Geometry check sheet. Reference: the model listing, model coordinates, mm. A direction names the side the tool comes from. Give positions to 0.01 mm unless a question says otherwise; leave off trailing zeros. Loops run counter-clockwise (first coordinate to the right, second up) from the corner with the lowest first, then second, coordinate; pieces in that order, holes last. Notation, with made-up numbers: (79, 88) -> (90, 88) arc R27 cw to (90, 116) -> close; hole circle Ø2 at (31, -14). An arc over 180 degrees is marked (long way). Answer as a JSON object with one key per item and string values.
from build123d import *

# Parameters (mm, degrees)
BASE_BLOCK_PROFILE_W        = 105
BASE_BLOCK_PROFILE_H        = 110
BASE_BLOCK_DEPTH            = 69
FORK_SLOT_PROFILE_W         = 105
FORK_SLOT_PROFILE_H         = 45
FORK_SLOT_CUT_DEPTH         = 60
FLANGE_CORNER_FILLETS_R15_R = 15
FLANGE_HOLES_PROFILE_R      = 7.5
FLANGE_HOLES_DEPTH          = 103.67545958
TOP_WINDOW_PROFILE_W        = 70
TOP_WINDOW_PROFILE_H        = 35
TOP_WINDOW_CUT_35X25_DEPTH  = 103.67545958
LUG_PLATE_A_DEPTH           = 10
LUG_START                   = 35
LUG_BOSS_A_PROFILE_R        = 17.5
LUG_BOSS_A_35_DEPTH         = 35
LUG_BORE_A_PROFILE_R        = 12
LUG_BORE_A_24_DEPTH         = 192.861929522
LUG_PLATE_B_DEPTH           = 10
LUG_BOSS_B_PROFILE_R        = 17.5
LUG_BOSS_B_35_DEPTH         = 35
LUG_BORE_B_PROFILE_R        = 12
LUG_BORE_B_24_DEPTH         = 245.782556568
LUG_BLEND_FILLETS_R5_R      = 5


with BuildPart() as part:
    # Base Block Profile → Base Block (new body)
    with BuildSketch(Plane(origin=(0, 0, 0), x_dir=(1, 0, 0), z_dir=(0, 1, 0))):
        Rectangle(BASE_BLOCK_PROFILE_W, BASE_BLOCK_PROFILE_H)
    extrude(amount=BASE_BLOCK_DEPTH)

    # Fork Slot Profile → Fork Slot Cut (cut)
    with BuildSketch(Plane.XY.offset(55)):
        with Locations((0, 34.5)):
            Rectangle(FORK_SLOT_PROFILE_W, FORK_SLOT_PROFILE_H)
    extrude(amount=-FORK_SLOT_CUT_DEPTH, mode=Mode.SUBTRACT)

    # Flange Corner Fillets R15
    flange_corner_fillets_r15_edges = [part.edges().sort_by_distance(p)[0] for p in [
        (52.5, 6, 55),
        (-52.5, 6, 55),
        (52.5, 63, 55),
        (-52.5, 63, 55),
    ]]
    fillet(flange_corner_fillets_r15_edges, radius=FLANGE_CORNER_FILLETS_R15_R)

    # Flange Holes Profile → Flange Holes (cut, through all)
    with BuildSketch(Plane(origin=(0, 69, 0), x_dir=(1, 0, 0), z_dir=(0, 1, 0))):
        with Locations(Location((-37.5, -40, 0), (0, 0, 270))):
            Circle(FLANGE_HOLES_PROFILE_R)
        with Locations(Location((37.5, -40, 0), (0, 0, 270))):
            Circle(FLANGE_HOLES_PROFILE_R)
    extrude(amount=-FLANGE_HOLES_DEPTH, mode=Mode.SUBTRACT)

    # Top Window Profile → Top Window Cut 35x25 (cut, through all)
    with BuildSketch(Plane(origin=(0, 69, 0), x_dir=(1, 0, 0), z_dir=(0, 1, 0))):
        with Locations((7.5, 27.5)):
            Rectangle(TOP_WINDOW_PROFILE_W, TOP_WINDOW_PROFILE_H)
    extrude(amount=-TOP_WINDOW_CUT_35X25_DEPTH, mode=Mode.SUBTRACT)

    # Lug Plate A Profile → Lug Plate A (add)
    with BuildSketch(Plane(origin=(0, 0, -55), x_dir=(-1, 0, 0), z_dir=(0, 0, -1))):
        with BuildLine():
            Line((-87.5, 0.5), (-52.5, 0))
            Line((-52.5, 0), (-52.5, 35.5))
            Line((-52.5, 35.5), (-87.5, 35.5))
            ThreePointArc((-87.5, 35.5), (-105, 18), (-87.5, 0.5))
        make_face()
    extrude(amount=-LUG_PLATE_A_DEPTH)

    # Lug Boss A Profile → Lug Boss A _35 (add)
    with BuildSketch(Plane(origin=(0, 0, -55), x_dir=(-1, 0, 0), z_dir=(0, 0, -1)).offset(LUG_START)):
        with Locations((-87.5, 18)):
            Circle(LUG_BOSS_A_PROFILE_R)
    extrude(amount=-LUG_BOSS_A_35_DEPTH)

    # Lug Bore A Profile → Lug Bore A _24 (cut, through all)
    with BuildSketch(Plane(origin=(0, 0, -90), x_dir=(-1, 0, 0), z_dir=(0, 0, -1))):
        with Locations((-87.5, 18)):
            Circle(LUG_BORE_A_PROFILE_R)
    extrude(amount=-LUG_BORE_A_24_DEPTH, mode=Mode.SUBTRACT)

    # Lug Plate B Profile → Lug Plate B (add)
    with BuildSketch(Plane.ZY.offset(52.5)):
        with BuildLine():
            Line((-55, 104), (-55, 69))
            Line((-55, 69), (-20, 69))
            Line((-20, 69), (-20, 104))
            ThreePointArc((-20, 104), (-37.5, 121.5), (-55, 104))
        make_face()
    extrude(amount=-LUG_PLATE_B_DEPTH)

    # Lug Boss B Profile → Lug Boss B _35 (add)
    with BuildSketch(Plane.ZY.offset(52.5).offset(LUG_START)):
        with Locations((-37.5, 104)):
            Circle(LUG_BOSS_B_PROFILE_R)
    extrude(amount=-LUG_BOSS_B_35_DEPTH)

    # Lug Bore B Profile → Lug Bore B _24 (cut, through all)
    with BuildSketch(Plane.ZY.offset(87.5)):
        with Locations((-37.5, 104)):
            Circle(LUG_BORE_B_PROFILE_R)
    extrude(amount=-LUG_BORE_B_24_DEPTH, mode=Mode.SUBTRACT)

    # Lug Blend Fillets R5
    lug_blend_fillets_r5_edges = [part.edges().sort_by_distance(p)[0] for p in [
        (-42.5, 69, -37.5),
        (52.5, 17.75, -45),
    ]]
    fillet(lug_blend_fillets_r5_edges, radius=LUG_BLEND_FILLETS_R5_R)


solid = part.part
1) Material ranges on line 1 along Z through (x, y) = (37, 62); line 2 along X through (y, z) = (66.5, 40); line 3 along Z through (x, y) = (-4.5, 39), recorded low to high. Write a range as from..to.
Geometry check:
{"line 1": "z = -55..-45, -10..32.52, 47.48..55", "line 2": "x = -52.5..-45, -30..30, 45..52.5", "line 3": "z = -55..-45, -10..-5"}
2) Draft check along X on faces 1 (the face through (-1, 6, 55)), 2 (the face through (7, 35, -10)), 3 (the face through (47.99, 63.08, 50.72)). Enter one of: pulls with the +X half, pulls with the -X half, needs draft (parallel to the pull), parting line crosses it, or undercut.
Geometry check:
{"face 1": "needs draft", "face 2": "undercut", "face 3": "pulls with the +X half"}
3) Tool access check on faces 4 (the face through (7, 35, -45)), 5 (the face through (-47, 86, -20)), 6 (the face through (-1, 35, -5)), 7 (the face through (-42.5, 88, -38)). Record the directions out of +Z, -Z, +X, -X, +Y, -Y that give a thin tool (end or side, any length) a straight path to the whole face; none if there is none.
Geometry check:
{"face 4": "+Y, -Y", "face 5": "+Z, +X, -X, +Y", "face 6": "+Z, +X, -X", "face 7": "+Z, -Z, +X, +Y"}
4) Section check C-C on z = -37.5. Record the cut outline in (x, y).
Geometry check:
{"outline": "(-87.5, 86.5) -> (-52.5, 86.5) -> (-52.5, 0) -> (-27.5, 0) -> (-27.5, 69) -> (-37.5, 69) arc R5 cw to (-42.5, 74) -> (-42.5, 92) -> (-87.5, 92) -> close; (-87.5, 116) -> (-42.5, 116) -> (-42.5, 121.5) -> (-87.5, 121.5) -> close; (42.5, 0) -> (52.5, 0) -> (52.5, 69) -> (42.5, 69) -> close"}
5) Section check A-A on z = 3.5. Record the cut outline in (x, y), plus the area to 3 significant figures.
Geometry check:
{"outline": "(-52.5, 0) -> (52.5, 0) -> (52.5, 12) -> (-52.5, 12) -> close; (-52.5, 57) -> (52.5, 57) -> (52.5, 69) -> (-52.5, 69) -> close", "area": "2,520 mm2"}
6) Section check B-B on x = 92. Record the cut outline in (y, z).
Geometry check:
{"outline": "(1.09, -90) -> (6.88, -90) -> (6.88, -45) -> (1.09, -45) -> close; (29.12, -90) -> (34.91, -90) -> (34.91, -45) -> (29.12, -45) -> close"}
7) Depth check by flat-ended pin: P1, Ø17, axis at x = 37.5, z = 40, coming from the +Y side; P2, Ø1, axis at x = 31.5, y = 47.5, coming from the +Z side; P3, Ø10, axis at x = -47.5, y = 85, coming from the +Z side. Enter the tip coordinate at first touch or a pass-through.
Geometry check:
{"P1": "stops at y = 69", "P2": "stops at z = -5", "P3": "stops at z = -20"}
8) Section check D-D on x = -34. Record the cut outline in (y, z).
Geometry check:
{"outline": "(0, -55) -> (69, -55) -> (69, 33.37) -> (57, 33.37) -> (57, -5) -> (12, -5) -> (12, 33.37) -> (0, 33.37) -> close; (0, 46.63) -> (12, 46.63) -> (12, 55) -> (0, 55) -> close; (57, 46.63) -> (69, 46.63) -> (69, 55) -> (57, 55) -> close"}
